Read the model definition and answer for the solid it produces. Units are mm, in the model's axes. A direction names the side the tool comes from. Coordinates: 2 decimals unless noted, no trailing zeros. Loops run counter-clockwise (first coordinate to the right, second up) from the corner with the lowest first, then second, coordinate; pieces in that order, holes last. Notation, with made-up numbers: M 81,-30.75 L 91,-30.75 A29 cw 91,8.25 Z; hole C 61.5,10 d5. An arc over 180 degrees is marked long. One line per item, written item: value. Start each with the question number.
1. Determine the mould class of faces 1 (the face through (20.39, 0.96, -17.13)), 2 (the face through (22, 12, 0)), 3 (the face through (21, 5, 28)) for opening direction Z: +Z half, -Z half, draft (parallel to the pull), parting line (faces both ways), or undercut.
2. For faces 4 (the face through (15, 0, 15)), 5 (the face through (18.68, 6.93, 16.72)), determine the directions among +Z, -Z, +X, -X, +Y, -Y from which every point of the face is accessible in a straight line to the end or side of a thin tool.
3. The part is cut by section A-A (x = 0). Write down the section's boundary in (y, z).
4. The part is cut by section B-B (y = 8). Write down the section's boundary in (x, z), then the cut area to 3 significant figures.
5. Flat-ended cylindrical pins translate along their axes: pin 1 (4 mm diameter, centred on x = 20.68, z = -17.36, fed in from -Y); pin 2 (1.5 mm diameter, centred on x = -6.5, y = 8, fed in from +Z); pin 3 (4 mm diameter, centred on x = 4, y = 9, fed in from +Z); pin 4 (2.5 mm diameter, centred on x = 20.68, z = 17.36, fed in from +Y). Find the tip coordinate at first contact, or state that the pin passes through.
6. Consider probe 1 along Z at (x, y) = (21, 4); probe 2 along Z at (x, y) = (0, 4.5); probe 3 along Z at (x, y) = (-26, 7.25). Determine where each line is inside the solid, lowest interval first.
```python
from build123d import *

# Parameters (mm, degrees)
SKETCH2_R             = 1.75
CUT_EXTRUDE1_DEPTH    = 10
M5_TAPPED_HOLE1_D     = 4.2
M5_TAPPED_HOLE1_DEPTH = 10
M5_TAPPED_HOLE1_TIP   = 1.2618073


with BuildPart() as part:
    # Sketch1 → Revolve1 (revolve)
    with BuildSketch(Plane(origin=(0, 0, 0), x_dir=(0, 0, -1), z_dir=(1, 0, 0))):
        Polygon((35, 10), (33, 12), (20, 12), (20, 0), (35, 0), align=None)
    revolve(axis=Axis((0, 0, 0), (0, 1, 0)))

    # Sketch2 → Cut-Extrude1 (cut)
    with BuildSketch(Plane(origin=(0, 12, 0), x_dir=(1, 0, 0), z_dir=(0, 1, 0))):
        with Locations(Location((-27, 0, 0), (0, 0, 270))):
            Circle(SKETCH2_R)
        with Locations(Location((-8.343458848, 25.67852594, 0), (0, 0, 270))):
            Circle(SKETCH2_R)
        with Locations(Location((-8.343458848, -25.67852594, 0), (0, 0, 90))):
            Circle(SKETCH2_R)
        with Locations(Location((20.683199964, 17.355265462, 0), (0, 0, 270))):
            Circle(SKETCH2_R)
        with Locations(Location((20.683199964, -17.355265462, 0), (0, 0, 90))):
            Circle(SKETCH2_R)
    extrude(amount=-CUT_EXTRUDE1_DEPTH, mode=Mode.SUBTRACT)

    # M5 Tapped Hole1
    with Locations(Plane(origin=(0, 12, 0), x_dir=(1, 0, 0), z_dir=(0, 1, 0))):
        with Locations((-27, 0), (-8.343458848, 25.67852594), (20.683199964, 17.355265462), (20.683199964, -17.355265462), (-8.343458848, -25.67852594)):
            Hole(M5_TAPPED_HOLE1_D / 2, depth=M5_TAPPED_HOLE1_DEPTH)
            with Locations((0, 0, -(M5_TAPPED_HOLE1_DEPTH + M5_TAPPED_HOLE1_TIP / 2))):  # 118° drill point
                Cone(0, M5_TAPPED_HOLE1_D / 2, M5_TAPPED_HOLE1_TIP, mode=Mode.SUBTRACT)


solid = part.part
```
Answer block:
1. face 1: undercut
1. face 2: draft
1. face 3: parting line
2. face 4: +Z, -Z, +X, -X, -Y
2. face 5: +Y
3. outline: M 0,-35 L 10,-35 L 12,-33 L 12,-20 L 0,-20 Z; M 0,20 L 12,20 L 12,33 L 10,35 L 0,35 Z
4. outline: C 0,0 d70; hole C -27,0 d4.2; hole C 0,0 d40; hole C -8.34,-25.68 d4.2; hole C -8.34,25.68 d4.2; hole C 20.68,-17.36 d4.2; hole C 20.68,17.36 d4.2
4. area: 2,520 mm2
5. pin 1: stops at y = 0
5. pin 2: stops at z = 34.52
5. pin 3: stops at z = 34.94
5. pin 4: stops at y = 1.49
6. probe 1: z = -28 to -19.43, -15.28 to 15.28, 19.43 to 28
6. probe 2: z = -35 to -20, 20 to 35
6. probe 3: z = -23.43 to -1.85, 1.85 to 23.43
